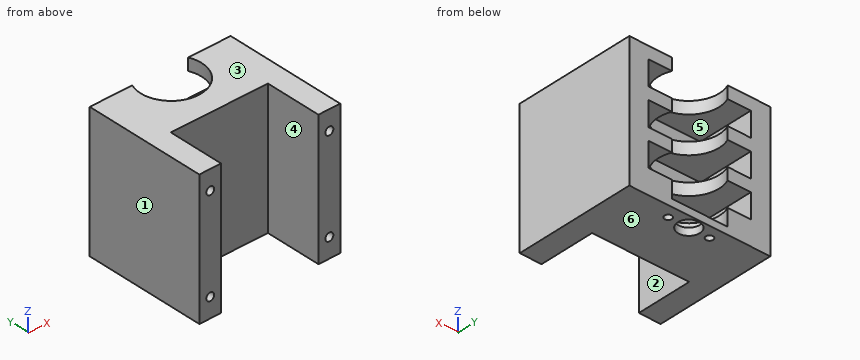
```python
from build123d import *

# Parameters (mm, degrees)
SKETCH1_W             = 58
SKETCH1_H             = 50
BOSS_EXTRUDE1_DEPTH   = 55
SKETCH3_R             = 4.5
SKETCH3_R_2           = 1.5
CUT_EXTRUDE2_DEPTH    = 5
SKETCH2_R             = 12.5
CUT_EXTRUDE1_DEPTH    = 52
SKETCH4_W             = 40
SKETCH4_H             = 46
CUT_EXTRUDE3_DEPTH    = 70
M4_TAPPED_HOLE1_D     = 3.3
M4_TAPPED_HOLE1_DEPTH = 10.1
M4_TAPPED_HOLE1_TIP   = 0.991420021
SKETCH8_W             = 42
SKETCH8_H             = 10
CUT_EXTRUDE4_DEPTH    = 23


with BuildPart() as part:
    # Sketch1 → Boss-Extrude1 (new body)
    with BuildSketch(Plane.XY):
        Rectangle(SKETCH1_W, SKETCH1_H)
    extrude(amount=BOSS_EXTRUDE1_DEPTH)

    # Sketch3 → Cut-Extrude2 (cut)
    with BuildSketch(Plane(origin=(0, 0, 0), x_dir=(-1, 0, 0), z_dir=(0, 0, -1))):
        with Locations((0, 20)):
            Circle(SKETCH3_R)
        with Locations((-8.5, 20)):
            Circle(SKETCH3_R_2)
        with Locations((8.5, 20)):
            Circle(SKETCH3_R_2)
    extrude(amount=-CUT_EXTRUDE2_DEPTH, mode=Mode.SUBTRACT)

    # Sketch2 → Cut-Extrude1 (cut)
    with BuildSketch(Plane.XY.offset(55)):
        with Locations((0, 20)):
            Circle(SKETCH2_R)
    extrude(amount=-CUT_EXTRUDE1_DEPTH, mode=Mode.SUBTRACT)

    # Sketch4 → Cut-Extrude3 (cut)
    with BuildSketch(Plane(origin=(0, 0, 0), x_dir=(-1, 0, 0), z_dir=(0, 0, -1))):
        with Locations((0, -25)):
            Rectangle(SKETCH4_W, SKETCH4_H)
    extrude(amount=-CUT_EXTRUDE3_DEPTH, mode=Mode.SUBTRACT)

    # M4 Tapped Hole1
    with Locations(Plane(origin=(0, -25, 0), x_dir=(-1, 0, 0), z_dir=(0, -1, 0))):
        with Locations((24.5, -47), (24.5, -8), (-24.5, -8), (-24.5, -47)):
            Hole(M4_TAPPED_HOLE1_D / 2, depth=M4_TAPPED_HOLE1_DEPTH)
            with Locations((0, 0, -(M4_TAPPED_HOLE1_DEPTH + M4_TAPPED_HOLE1_TIP / 2))):  # 118° drill point
                Cone(0, M4_TAPPED_HOLE1_D / 2, M4_TAPPED_HOLE1_TIP, mode=Mode.SUBTRACT)

    # Sketch8 → Cut-Extrude4 (cut)
    with BuildSketch(Plane(origin=(0, 25, 0), x_dir=(1, 0, 0), z_dir=(0, 1, 0))):
        with Locations((0, -15)):
            Rectangle(SKETCH8_W, SKETCH8_H)
        with Locations((0, -30)):
            Rectangle(SKETCH8_W, SKETCH8_H)
        with Locations((0, -45)):
            Rectangle(SKETCH8_W, SKETCH8_H)
    extrude(amount=-CUT_EXTRUDE4_DEPTH, mode=Mode.SUBTRACT)


solid = part.part
```
Read the model definition and answer for the solid it produces. Units are mm, in the model's axes. Face numbers are marked on the shaded views. A direction names the side the tool comes from. Round coordinates to 2 decimals unless told otherwise and drop trailing zeros. Write each loop counter-clockwise with the first axis right and the second up, starting at its lowest first coordinate (ties: lowest second). Pieces come first, ordered by that corner, then holes. Notation, with made-up numbers: M -20,-19.75 L -8,-19.75 A15 ccw -8,-6.75 Z; hole C 24,-17 d6. An arc over 180 degrees is marked long. One line per item, written item: value.
Q1. For a pull along X with two mould halves and no side action, classify the marked faces 1, 2 and 3 as +X half, -X half, draft (parallel to the pull), parting line (faces both ways), or undercut.
Data:
face 1: -X half
face 2: undercut
face 3: draft
Q2. Find section B-B on x = 0. Write down the section's boundary in (y, z), plus the area to 3 significant figures.
Data:
outline: M -2,0 L 15.5,0 L 15.5,3 L 7.5,3 L 7.5,10 L 2,10 L 2,20 L 7.5,20 L 7.5,25 L 2,25 L 2,35 L 7.5,35 L 7.5,40 L 2,40 L 2,50 L 7.5,50 L 7.5,55 L -2,55 Z; M 24.5,0 L 25,0 L 25,3 L 24.5,3 Z
area: 383 mm2
Q3. Flat-ended cylindrical pins translate along their axes: pin 1 Ø5 at (x, y) = (8.5, 20) entering from +Z; pin 2 Ø2 at (x, z) = (-2.5, 22.5) entering from +Y; pin 3 Ø2 at (x, z) = (5.5, 35) entering from -Y. Find the tip coordinate at first contact, or state that the pin passes through.
Data:
pin 1: z = 3
pin 2: y = 8
pin 3: y = -2
Q4. Find section D-D on x = 19. Write down the section's boundary in (y, z).
Data:
outline: M -2,0 L 25,0 L 25,10 L 2,10 L 2,20 L 25,20 L 25,25 L 2,25 L 2,35 L 25,35 L 25,40 L 2,40 L 2,50 L 25,50 L 25,55 L -2,55 Z
Q5. Straight lines are drawn through the part: line 1 (Z direction, x = -24.5, y = -19.25); line 2 (X direction, y = -19.25, z = 8); line 3 (Z direction, x = 13, y = 6). For each, find the intervals that lie inside material, in ascending order. Write a range as [from, to].
Data:
line 1: [0, 6.35], [9.65, 45.35], [48.65, 55]
line 2: [-29, -26.15], [-22.85, -20], [20, 22.85], [26.15, 29]
line 3: [0, 10], [20, 25], [35, 40], [50, 55]
Q6. Find section C-C on z = 28. Write down the section's boundary in (x, y), plus the area to 3 significant figures.
Data:
outline: M -29,-25 L -20,-25 L -20,-2 L 20,-2 L 20,-25 L 29,-25 L 29,25 L 21,25 L 21,2 L -21,2 L -21,25 L -29,25 Z
area: 1,010 mm2
Q7. Find section A-A on y = -3.5. Write down the section's boundary in (x, z), plus the area to 3 significant figures.
Data:
outline: M -29,0 L -20,0 L -20,55 L -29,55 Z; M 20,0 L 29,0 L 29,55 L 20,55 Z
area: 990 mm2
Q8. Which of the six approach directions +Z, -Z, +X, -X, +Y, -Y give full straight-line access (tool end or side, diameter ignored) to the marked faces 4, 5 and 6?
Data:
face 4: +Z, -Z, -Y
face 5: +Y
face 6: -Z, +X, -X, +Y, -Y
